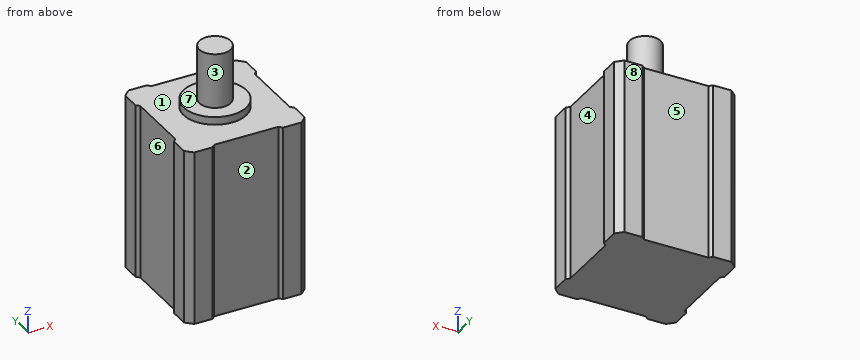
from build123d import *

# Parameters (mm, degrees)
SKETCH1_W           = 77
SKETCH1_H           = 77
EXTRUDE1_DEPTH      = 112
SKETCH3_R           = 58.910335971
SKETCH3_R_2         = 51.5
EXTRUDE3_DEPTH      = 125.533128123
EXTRUDE7_DEPTH      = 125.533128123
SKETCH2_R           = 10
EXTRUDE10_DEPTH     = 80
CIRPATTERN3_COUNT   = 4
EXTRUDE13_START     = 5
SKETCH11_R          = 20
SKETCH11_R_2        = 10
EXTRUDE13_DEPTH     = 5
BOSS_EXTRUDE1_START = 120
SKETCH12_R          = 10
BOSS_EXTRUDE1_DEPTH = 120
SCALE1_SCALE        = 0.55


with BuildPart() as part:
    # Sketch1 → Extrude1 (new body)
    with BuildSketch(Plane.XY):
        Rectangle(SKETCH1_W, SKETCH1_H)
    extrude(amount=EXTRUDE1_DEPTH)

    # Sketch3 → Extrude3 (cut, through all)
    with BuildSketch(Plane.XY.offset(112)):
        Circle(SKETCH3_R)
        Circle(SKETCH3_R_2, mode=Mode.SUBTRACT)
    extrude(amount=-EXTRUDE3_DEPTH, mode=Mode.SUBTRACT)

    # Sketch7 → Extrude7 (cut, through all)
    with BuildSketch(Plane.XY.offset(112)):
        Polygon((-22.5, 38.5), (22.5, 38.5), (20.5, 36.5), (-20.5, 36.5), align=None)
    extrude7 = extrude(amount=-EXTRUDE7_DEPTH, mode=Mode.SUBTRACT)

    # Sketch2 → Extrude10 (cut)
    with BuildSketch(Plane.XY.offset(112)):
        Circle(SKETCH2_R)
    extrude(amount=-EXTRUDE10_DEPTH, mode=Mode.SUBTRACT)

    # CirPattern3: Extrude7 ×4 about axis
    cirpattern3_axis = Axis((0, 0, 0), (0, 0, 1))
    for i in range(1, CIRPATTERN3_COUNT):
        add(extrude7.rotate(cirpattern3_axis, i * 360 / CIRPATTERN3_COUNT), mode=Mode.SUBTRACT)

    # Sketch11 → Extrude13 (add)
    with BuildSketch(Plane.XY.offset(112).offset(EXTRUDE13_START)):
        Circle(SKETCH11_R)
        Circle(SKETCH11_R_2, mode=Mode.SUBTRACT)
    extrude(amount=-EXTRUDE13_DEPTH)

    # Sketch12 → Boss-Extrude1 (add)
    with BuildSketch(Plane.XY.offset(32).offset(BOSS_EXTRUDE1_START)):
        Circle(SKETCH12_R)
    extrude(amount=-BOSS_EXTRUDE1_DEPTH)


with BuildPart() as part_1:
    # Scale1: scaled about (0, 0, 57.926521071)
    add(part.part.scale(SCALE1_SCALE).moved(Location((0, 0, 26.066934482))))


solid = part_1.part
Verification items for the finished model (mm, model axes). Face numbers are marked on the shaded views. A direction names the side the tool comes from. Give positions to 0.01 mm unless a question says otherwise; leave off trailing zeros. Write each loop counter-clockwise with the first axis right and the second up, starting at its lowest first coordinate (ties: lowest second). Pieces come first, ordered by that corner, then holes. Notation, with made-up numbers: M 14.5,8.25 L 54.5,8.25 A8 cw 54.5,17.25 Z; hole C 82,51 d4. An arc over 180 degrees is marked long. Put each result on its own line as item: value. Start each with the question number.
1. Section check C-C (y = 3). Record the cut outline in (x, z) (3 decimals).
2. Section check B-B (x = 0). Record the cut outline in (y, z) (3 decimals), and give its area (3 significant figures).
3. Set-up check for the marked faces 5, 6, 7 and 8: record each of +Z, -Z, +X, -X, +Y, -Y from which the full face is reachable in a straight line by a thin tool's end or side.
4. Section check D-D (y = -15.5). Record the cut outline in (x, z) (3 decimals), and give its area (3 significant figures).
5. Scan lines: line 1 along Z through (x, y) = (16, -18.5); line 2 along X through (y, z) = (9, 36) (3 decimals). Record each from-to range of solid material in increasing order. Write a range as [from, to].
6. Draft check along Y on the marked faces 1, 2, 3 and 4. Enter one of: +Y half, -Y half, draft (parallel to the pull), parting line (faces both ways), or undercut.
7. Go/stop test with flat-tipped pins: pin 1 Ø10 at (x, y) = (4, 12) entering from +Z; pin 2 Ø7 at (y, z) = (2, 72) entering from +X (3 decimals); pin 3 Ø12 at (x, z) = (4, 56) entering from -Y (3 decimals). Record where each tip stops, or that it passes through.
8. Section check A-A (z = 57.5). Record the cut outline in (x, y) (3 decimals), and give its area (3 significant figures).
Answer list:
1. outline: M -20.075,26.067 L 20.075,26.067 L 20.075,87.667 L 10.583,87.667 L 10.583,90.417 L 4.61,90.417 L 4.61,109.667 L -4.61,109.667 L -4.61,90.417 L -10.583,90.417 L -10.583,87.667 L -20.075,87.667 Z
2. outline: M -20.075,26.067 L 20.075,26.067 L 20.075,87.667 L 11,87.667 L 11,90.417 L 5.5,90.417 L 5.5,109.667 L -5.5,109.667 L -5.5,90.417 L -11,90.417 L -11,87.667 L -20.075,87.667 Z
2. area: 2,750 mm2
3. face 5: +Z, -Z, +Y
3. face 6: +Z, -Z, -X
3. face 7: +Z
3. face 8: +Z, -Z, +X, -X, +Y
4. outline: M -21.175,26.067 L 21.175,26.067 L 21.175,87.667 L -21.175,87.667 Z
4. area: 2,610 mm2
5. line 1: [26.07, 87.67]
5. line 2: [-20.075, 20.075]
6. face 1: draft
6. face 2: -Y half
6. face 3: parting line
6. face 4: undercut
7. pin 1: z = 90.42
7. pin 2: x = 20.075
7. pin 3: y = -20.075
8. outline: M -21.175,-18.813 A28.325 ccw -18.813,-21.175 L -12.375,-21.175 L -11.275,-20.075 L 11.275,-20.075 L 12.375,-21.175 L 18.813,-21.175 A28.325 ccw 21.175,-18.813 L 21.175,-12.375 L 20.075,-11.275 L 20.075,11.275 L 21.175,12.375 L 21.175,18.813 A28.325 ccw 18.813,21.175 L 12.375,21.175 L 11.275,20.075 L -11.275,20.075 L -12.375,21.175 L -18.813,21.175 A28.325 ccw -21.175,18.813 L -21.175,12.375 L -20.075,11.275 L -20.075,-11.275 L -21.175,-12.375 Z
8. area: 1,680 mm2
